Job drawing, mm, ordinate dimensions from the low corner. One solid piece. Coordinates: 2 decimals unless noted, no trailing zeros. Order: outer loops, then holes, each group sorted by start corner. A loop starts at its lowest first (then second) coordinate and runs counter-clockwise, first axis right, second up. Notation, with made-up numbers: M 10.5,17.5 L 54.5,17.5 A25 ccw 54.5,39.5 Z; hole C 40.25,23.5 d4. An arc over 180 degrees is marked long. Write item = value, one per line.
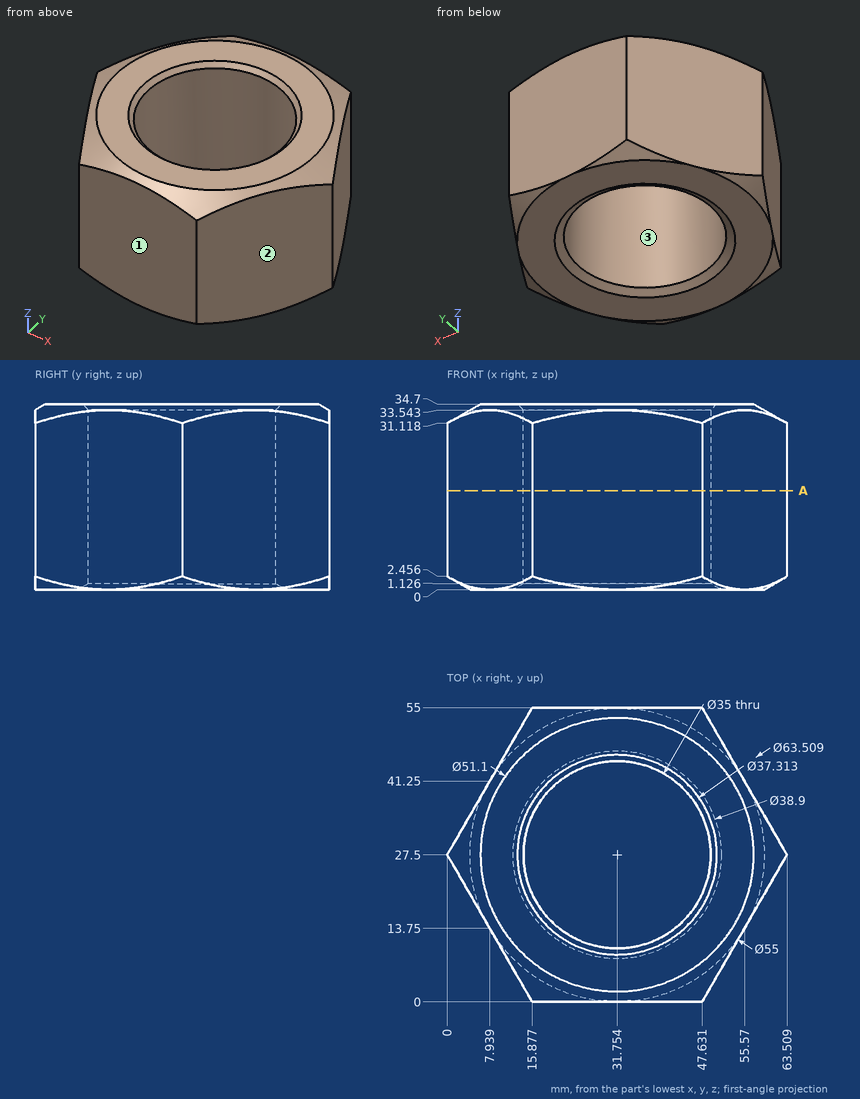
(1) Pin check, flat tips, straight feed: pin 1 Ø5 at (x, y) = (44, 16) entering from -Z; pin 2 Ø12 at (y, z) = (40, 15) entering from +X (1 decimal). Stop position of each tip, or through.
Evaluation:
pin_1 = 0.09
pin_2 = 59.8
(2) Pull direction X, two halves, no side cores. Call the marked faces 1, 2 and 3: +X half, -X half, draft (parallel to the pull), parting line (faces both ways), or undercut.
Evaluation:
face_1 = draft
face_2 = +X half
face_3 = undercut
(3) Wall check: line 1 (Y direction, x = 31.5, z = 26.5); line 2 (Y direction, x = 20.5, z = 2); line 3 (X direction, y = 34.5, z = 4) (1 decimal). Give the ranges that are in metal, low to high. Write a range as from..to.
Evaluation:
line_1 = 0..10, 45..55
line_2 = 0..14.1, 40.9..55
line_3 = 4..15.7, 47.8..59.5
(4) Slice it at A-A, the plane z = 18.5. Write the cut outline in (x, y) (1 decimal), then the cut area to 3 significant figures.
Evaluation:
outline = M 0,27.5 L 15.9,0 L 47.6,0 L 63.5,27.5 L 47.6,55 L 15.9,55 Z; hole C 31.8,27.5 d35
area = 1,660 mm²
